Check sheet for the modelled part. Datum: model origin and axes. Units: mm. A direction names the side the tool comes from. Give positions to 0.01 mm unless a question says otherwise; leave off trailing zeros. Write each loop counter-clockwise with the first axis right and the second up, starting at its lowest first coordinate (ties: lowest second). Pieces come first, ordered by that corner, then holes. Notation, with made-up numbers: M 20,3 L 65,3 A16 cw 65,32 Z; hole C -39,59.25 d3. An arc over 180 degrees is marked long. Write item = value, one per line. Start each with the question number.
1) Access from +Z, -Z, +X, -X, +Y, -Y to the whole of each face (thin tool, end or side, straight path). Record for faces 4 (the flat face through (-49, 1.9, 0)), 5 (the flat face through (-1, 5, 0)).
2) Scan lines: line 1 along X through (y, z) = (3, 0); line 2 along X through (y, z) = (4.65, -1.5); line 3 along Z through (x, y) = (-50, 4.6). Record each from-to range of solid material in increasing order. Write a range as [from, to].
3) Mould release check, pull along Z, two halves, no side actions. Record for faces 1 (the flat face through (55, 2, 0)), 2 (the flat face through (-1, 2, 5)), 3 (the flat face through (49, 1.9, 0)): released by +Z, released by -Z, zero draft, split by the parting line, or undercut.
4) Cross-section at C-C, the plane z = 0. Record the cut outline in (x, y), plus the area to 3 significant figures.
5) Go/stop test with a flat-tipped pin: pin 1 (1.8 mm diameter, centred on x = -48, z = -1.5, fed in from +Y). Record where the tip stops, or that it passes through.
6) Cross-section at B-B, the plane y = 3.75. Record the cut outline in (x, z).
7) Cross-section at A-A, the plane x = -49. Record the cut outline in (y, z).
```python
from build123d import *

# Parameters (mm, degrees)
SKETCH1_W           = 110
SKETCH1_H           = 10
BOSS_EXTRUDE1_DEPTH = 5
SKETCH2_R           = 3
CUT_EXTRUDE1_DEPTH  = 3.1


with BuildPart() as part:
    # Sketch1 → Boss-Extrude1 (new body)
    with BuildSketch(Plane(origin=(0, 0, 0), x_dir=(1, 0, 0), z_dir=(0, 1, 0))):
        Rectangle(SKETCH1_W, SKETCH1_H)
    extrude(amount=BOSS_EXTRUDE1_DEPTH)

    # Sketch2 → Cut-Extrude1 (cut)
    with BuildSketch(Plane(origin=(0, 5, 0), x_dir=(1, 0, 0), z_dir=(0, 1, 0))):
        with Locations(Location((-49, 0, 0), (0, 0, 270))):
            Circle(SKETCH2_R)
        with Locations(Location((49, 0, 0), (0, 0, 270))):
            Circle(SKETCH2_R)
    extrude(amount=-CUT_EXTRUDE1_DEPTH, mode=Mode.SUBTRACT)


solid = part.part
```
Reply:
q1.face_4 = +Y
q1.face_5 = +Z, -Z, +X, -X, +Y
q2.line_1 = [-55, -52], [-46, 46], [52, 55]
q2.line_2 = [-55, -51.6], [-46.4, 46.4], [51.6, 55]
q2.line_3 = [-5, -2.83], [2.83, 5]
q3.face_1 = zero draft
q3.face_2 = released by +Z
q3.face_3 = undercut
q4.outline = M -55,0 L 55,0 L 55,5 L 52,5 L 52,1.9 L 46,1.9 L 46,5 L -46,5 L -46,1.9 L -52,1.9 L -52,5 L -55,5 Z
q4.area = 513 mm2
q5.pin_1 = 1.9
q6.outline = M -55,-5 L 55,-5 L 55,5 L -55,5 Z; hole C -49,0 d6; hole C 49,0 d6
q7.outline = M 0,-5 L 5,-5 L 5,-3 L 1.9,-3 L 1.9,3 L 5,3 L 5,5 L 0,5 Z
